from build123d import *

# Parameters (mm, degrees)
SKETCH4_R          = 7
CUT_EXTRUDE1_DEPTH = 8.5
SKETCH5_R          = 4.25
CUT_EXTRUDE2_DEPTH = 8.5


with BuildPart() as part:
    # Sketch2 → Revolve1 (revolve)
    with BuildSketch(Plane.XY, mode=Mode.PRIVATE) as revolve1_sk:
        Polygon((-80.999754507, 110), (-80.999754507, 100), (-70.999754507, 100), (-70.999754507, 105), (-63.499754507, 105), (-63.499754507, 100), (-53.999754507, 100), (-53.999754507, 100.5), (69.000245493, 100.5), (69.000245493, 100), (119.000245493, 100), (119.000245493, 110), align=None)
    revolve(revolve1_sk.sketch.rotate(Axis((-113.629726069, 0, 0), (1, 0, 0)), 90), axis=Axis((-113.629726069, 0, 0), (1, 0, 0)))

    # Sketch4 → Cut-Extrude1 (cut)
    with BuildSketch(Plane(origin=(0, 110, 0), x_dir=(1, 0, 0), z_dir=(0, 1, 0))):
        with Locations(Location((106.500245493, 0, 0), (0, 0, 270))):
            Circle(SKETCH4_R)
    extrude(amount=-CUT_EXTRUDE1_DEPTH, mode=Mode.SUBTRACT)

    # Sketch5 → Cut-Extrude2 (cut)
    with BuildSketch(Plane(origin=(0, 101.5, 0), x_dir=(1, 0, 0), z_dir=(0, 1, 0))):
        with Locations(Location((106.500245493, 0, 0), (0, 0, 270))):
            Circle(SKETCH5_R)
    extrude(amount=-CUT_EXTRUDE2_DEPTH, mode=Mode.SUBTRACT)


solid = part.part
Here's how the part is built. I have some questions about the finished solid (model axes, mm). A direction names the side the tool comes from. Coordinates: 2 decimals unless noted, no trailing zeros. Loops run counter-clockwise (first coordinate to the right, second up) from the corner with the lowest first, then second, coordinate; pieces in that order, holes last.
1. Imagine slicing it at B-B, the plane y = -11. Please give me the cut outline in (x, z).
2. Imagine slicing it at D-D, the plane x = 92.5. Please give me the cut outline in (y, z), and give its area (3 significant figures).
3. If we mould it in two halves opening along Y, with no side actions, what happens to faces 1 (the cylindrical face through (94.35, -30.04, 95.38)), 2 (the flat face through (-81, 97.3, 23.9)), 3 (the flat face through (103, 101.5, 3))? For each: pulls with the +Y half, pulls with the -Y half, needs draft (parallel to the pull), parting line crosses it, or undercut.
4. I need wall thicknesses on L1, parallel to Z at x = 72.5, y = 3.5; L2, parallel to X at y = 100.65, z = 0; L3, parallel to X at y = 107, z = 0. Which ranges of each line are inside material? Lowest first, please.
5. For faces 4 (the cylindrical face through (17.6, 97.59, 50.76)), 5 (the cylindrical face through (-67.2, -31.54, 100.15)), 6 (the cylindrical face through (113.44, 105.81, -0.91)), which set-ups out of +Z, -Z, +X, -X, +Y, -Y let a thin tool reach every point of the face, with its end or its side?
6. For P1, Ø2, axis at x = -13, y = 36.5, coming from the +Z side; P2, Ø12, axis at y = -87.5, z = -79, coming from the +X side; P3, Ø10, axis at x = -31, y = -16, coming from the -Z side; P4, Ø1, axis at x = -32.5, z = 30.5, coming from the +Y side, each with a flat end and sliding along its axis, tell me the tip position at first contact or that it passes through.
7. Imagine slicing it at A-A, the plane z = 0. Count the separate pieces of the cut face and the enclosed holes in it, and give its area (3 significant figures).
8. Imagine slicing it at C-C, the plane z = 29. Please give me the cut outline in (x, y) (3 decimals).
Taken from the geometry:
1. outline: (-81, -109.45) - (119, -109.45) - (119, -99.39) - (69, -99.39) - (69, -99.9) - (-54, -99.9) - (-54, -99.39) - (-63.5, -99.39) - (-63.5, -104.42) - (-71, -104.42) - (-71, -99.39) - (-81, -99.39) - close; (-81, 99.39) - (-71, 99.39) - (-71, 104.42) - (-63.5, 104.42) - (-63.5, 99.39) - (-54, 99.39) - (-54, 99.9) - (69, 99.9) - (69, 99.39) - (119, 99.39) - (119, 109.45) - (-81, 109.45) - close
2. outline: circle Ø220 at (0, 0); hole circle Ø200 at (0, 0)
2. area: 6,600 mm2
3. face 1: undercut
3. face 2: needs draft
3. face 3: pulls with the +Y half
4. L1: z = -109.94 to -99.94, 99.94 to 109.94
4. L2: x = -81 to -71, -63.5 to 102.25, 110.75 to 119
4. L3: x = -81 to 99.5, 113.5 to 119
5. face 4: +X, -X
5. face 5: none
5. face 6: +Y
6. P1: stops at z = 104.11
6. P2: passes through
6. P3: stops at z = -109.45
6. P4: stops at y = 105.83
7. separate pieces: 3
7. enclosed holes: 0
7. area: 3,670 mm2
8. outline: (-81, -106.108) - (119, -106.108) - (119, -95.703) - (69, -95.703) - (69, -96.225) - (-54, -96.225) - (-54, -95.703) - (-63.5, -95.703) - (-63.5, -100.916) - (-71, -100.916) - (-71, -95.703) - (-81, -95.703) - close; (-81, 95.703) - (-71, 95.703) - (-71, 100.916) - (-63.5, 100.916) - (-63.5, 95.703) - (-54, 95.703) - (-54, 96.225) - (69, 96.225) - (69, 95.703) - (119, 95.703) - (119, 106.108) - (-81, 106.108) - close
